```python
from build123d import *

# Parameters (mm, degrees)
SKETCH1_R           = 15
SKETCH1_R_2         = 12.5
BOSS_EXTRUDE1_DEPTH = 5
SKETCH2_R           = 15
SKETCH2_R_2         = 12.5
BOSS_EXTRUDE2_DEPTH = 10
SKETCH3_R           = 20
SKETCH3_R_2         = 14.885772681
BOSS_EXTRUDE5_DEPTH = 3
SKETCH6_R           = 1.03
CUT_EXTRUDE9_DEPTH  = 10


with BuildPart() as part:
    # Sketch1 → Boss-Extrude1 (new body)
    with BuildSketch(Plane.XY):
        Circle(SKETCH1_R)
        Circle(SKETCH1_R_2, mode=Mode.SUBTRACT)
    extrude(amount=BOSS_EXTRUDE1_DEPTH)

    # Sketch2 → Boss-Extrude2 (add)
    with BuildSketch(Plane.XY.offset(5)):
        Circle(SKETCH2_R)
        Circle(SKETCH2_R_2, mode=Mode.SUBTRACT)
    extrude(amount=BOSS_EXTRUDE2_DEPTH)

    # Sketch3 → Boss-Extrude5 (add)
    with BuildSketch(Plane.XY.offset(12)):
        Circle(SKETCH3_R)
        Circle(SKETCH3_R_2, mode=Mode.SUBTRACT)
    extrude(amount=BOSS_EXTRUDE5_DEPTH)

    # Sketch6 → Cut-Extrude9 (cut)
    with BuildSketch(Plane.XY.offset(15)):
        with Locations((17.988559183, 0.641668533)):
            Circle(SKETCH6_R)
        with Locations((13.173560353, -12.266104012)):
            Circle(SKETCH6_R)
        with Locations((0.641668533, -17.988559183)):
            Circle(SKETCH6_R)
        with Locations((-12.266104012, -13.173560353)):
            Circle(SKETCH6_R)
        with Locations((-17.988559183, -0.641668533)):
            Circle(SKETCH6_R)
        with Locations((-13.173560353, 12.266104012)):
            Circle(SKETCH6_R)
        with Locations((-0.641668533, 17.988559183)):
            Circle(SKETCH6_R)
        with Locations((12.266104012, 13.173560353)):
            Circle(SKETCH6_R)
    extrude(amount=-CUT_EXTRUDE9_DEPTH, mode=Mode.SUBTRACT)


solid = part.part
```
Design review of the part built by this model. Coordinates are the model's own, in mm. Give positions to 0.01 mm unless a question says otherwise; leave off trailing zeros. Write each loop counter-clockwise with the first axis right and the second up, starting at its lowest first coordinate (ties: lowest second). Pieces come first, ordered by that corner, then holes.
(1) Wall thickness on line 1 along X through (y, z) = (-1.5, 14.25); line 2 along Z through (x, y) = (-4, 15.5); line 3 along Y through (x, z) = (6.5, 10.75): over which ranges is each line inside the solid? List them lowest first.
Checked values:
line 1: x = -19.94 to -18.56, -17.42 to -12.41, 12.41 to 19.94
line 2: z = 12 to 15
line 3: y = -13.52 to -10.68, 10.68 to 13.52
(2) Add section D-D (z = 7). Give the boundary of the cut face in (x, y), and give its area (3 significant figures).
Checked values:
outline: circle Ø30 at (0, 0); hole circle Ø25 at (0, 0)
area: 216 mm2
(3) Clearance check with flat-ended pins moving along their axes: pin 1 Ø2.5 at (x, y) = (-12.27, -13.17) entering from -Z; pin 2 Ø6 at (x, z) = (14.5, 7.5) entering from -Y; pin 3 Ø3 at (x, z) = (-14, 9.5) entering from -Y; pin 4 Ø1.9 at (x, y) = (-0.64, 17.99) entering from +Z. State where each tip first meets the part, or that it passes through.
Checked values:
pin 1: stops at z = 12
pin 2: stops at y = -9.63
pin 3: stops at y = -8.29
pin 4: passes through
(4) Add section B-B (y = -8). Give the boundary of the cut face in (x, z).
Checked values:
outline: (-18.33, 12) - (-12.69, 12) - (-12.69, 0) - (-9.6, 0) - (-9.6, 15) - (-18.33, 15) - close; (9.6, 0) - (12.69, 0) - (12.69, 12) - (18.33, 12) - (18.33, 15) - (9.6, 15) - close
(5) Add section C-C (x = -1). Give the boundary of the cut face in (y, z).
Checked values:
outline: (-19.97, 12) - (-14.97, 12) - (-14.97, 0) - (-12.46, 0) - (-12.46, 15) - (-19.97, 15) - close; (12.46, 0) - (14.97, 0) - (14.97, 12) - (17.02, 12) - (17.02, 15) - (12.46, 15) - close; (18.95, 12) - (19.97, 12) - (19.97, 15) - (18.95, 15) - close
(6) Add section A-A (x = 6). Give the boundary of the cut face in (y, z).
Checked values:
outline: (-19.08, 12) - (-13.75, 12) - (-13.75, 0) - (-10.97, 0) - (-10.97, 15) - (-19.08, 15) - close; (10.97, 0) - (13.75, 0) - (13.75, 12) - (19.08, 12) - (19.08, 15) - (10.97, 15) - close
(7) Mouldability with a two-part tool opening along X and no side actions: class faces 1 (the face through (-5, -15, 12)), 2 (the face through (-13.4, 11.26, 13.52)), 3 (the face through (-14.985, 0.66, 5.916)) as +X half, -X half, draft (parallel to the pull), parting line (faces both ways), or undercut.
Checked values:
face 1: draft
face 2: undercut
face 3: parting line
